from build123d import *

# Parameters (mm, degrees)
BASE_PLATE_DEPTH         = 60
MOUNTING_HOLES_SKETCH_R  = 5
MOUNTING_HOLES_DEPTH     = 60
EYE_UPRIGHT_PROFILE_R    = 12.5
EYE_UPRIGHT_DEPTH        = 10
UPRIGHT_ROOT_FILLET_R6_R = 6


with BuildPart() as part:
    # Base Plate Profile → Base Plate (new body)
    with BuildSketch(Plane.XY):
        Polygon((0, 0), (50, 0), (42, -8), (60, -8), (60, 8), (-60, 8), (-60, -8), (-42, -8), (-50, 0), align=None)
    extrude(amount=-BASE_PLATE_DEPTH)

    # Mounting Holes Sketch → Mounting Holes (cut)
    with BuildSketch(Plane(origin=(0, 8, 0), x_dir=(1, 0, 0), z_dir=(0, 1, 0))):
        with Locations(Location((34, 45, 0), (0, 0, 180))):
            Circle(MOUNTING_HOLES_SKETCH_R)
        with Locations(Location((34, 15, 0), (0, 0, 180))):
            Circle(MOUNTING_HOLES_SKETCH_R)
        with Locations(Location((-34, 45, 0), (0, 0, 180))):
            Circle(MOUNTING_HOLES_SKETCH_R)
        with Locations(Location((-34, 15, 0), (0, 0, 180))):
            Circle(MOUNTING_HOLES_SKETCH_R)
    extrude(amount=-MOUNTING_HOLES_DEPTH, mode=Mode.SUBTRACT)

    # Eye Upright Profile → Eye Upright (add, symmetric)
    with BuildSketch(Plane(origin=(0, 0, 0), x_dir=(0, 0, -1), z_dir=(1, 0, 0))):
        with BuildLine():
            Line((0, 8), (0, 34))
            ThreePointArc((0, 34), (30, 64), (60, 34))
            Line((60, 34), (60, 8))
            Line((60, 8), (0, 8))
        make_face()
        with Locations((30, 34)):
            Circle(EYE_UPRIGHT_PROFILE_R, mode=Mode.SUBTRACT)
    extrude(amount=EYE_UPRIGHT_DEPTH, both=True)

    # Upright Root Fillet R6
    upright_root_fillet_r6_edges = [part.edges().sort_by_distance(p)[0] for p in [
        (-60, 8, -30),
        (60, 8, -30),
        (10, 8, -30),
        (-10, 8, -30),
    ]]
    fillet(upright_root_fillet_r6_edges, radius=UPRIGHT_ROOT_FILLET_R6_R)


solid = part.part
Design review of the part built by this model. Coordinates are the model's own, in mm. A direction names the side the tool comes from. Give positions to 0.01 mm unless a question says otherwise; leave off trailing zeros. Loops run counter-clockwise (first coordinate to the right, second up) from the corner with the lowest first, then second, coordinate; pieces in that order, holes last. Notation, with made-up numbers: M -29,75 L 20,75 A18 ccw 20,80 Z; hole C -33,-38.5 d8. An arc over 180 degrees is marked long. Answer as a JSON object with one key per item and string values.
Item 1: Wall thickness on line 1 along Z through (x, y) = (-34, 2); line 2 along Z through (x, y) = (4.5, 34.5); line 3 along X through (y, z) = (6.5, -18): over which ranges is each line inside the solid? List them lowest first.
Output values:
{"line 1": "z = -60 to -50, -40 to -20, -10 to 0", "line 2": "z = -60 to -42.49, -17.51 to 0", "line 3": "x = -57.97 to -38, -30 to 30, 38 to 57.97"}
Item 2: Mouldability with a two-part tool opening along X and no side actions: class faces 1 (the face through (-60, -3, -30)), 2 (the face through (0.14, 63.993, -29.34)), 3 (the face through (46, -4, -30)), 4 (the face through (-46, -4, -30)) as pulls with the +X half, pulls with the -X half, needs draft (parallel to the pull), parting line crosses it, or undercut.
Output values:
{"face 1": "pulls with the -X half", "face 2": "needs draft", "face 3": "undercut", "face 4": "undercut"}
Item 3: For P1, Ø25, axis at y = 41.5, z = -37, coming from the +X side; P2, Ø3, axis at x = 43.5, z = -31, coming from the +Y side; P3, Ø10, axis at x = 11.5, z = -29, coming from the -Y side; P4, Ø1.5, axis at x = 1, y = 10.5, coming from the +Z side, all flat-tipped, find the tip position at first contact; note any pin that passes through.
Output values:
{"P1": "stops at x = 10", "P2": "stops at y = 8", "P3": "stops at y = 0", "P4": "stops at z = 0"}
Item 4: We need section A-A (z = -30). State the section outline as (x, y) points.
Output values:
{"outline": "M -60,-8 L -42,-8 L -50,0 L 50,0 L 42,-8 L 60,-8 L 60,2 A6 ccw 54,8 L 16,8 A6 cw 10,14 L 10,21.5 L -10,21.5 L -10,14 A6 cw -16,8 L -54,8 A6 ccw -60,2 Z; M -10,46.5 L 10,46.5 L 10,64 L -10,64 Z"}
Item 5: We need section D-D (x = -48). State the section outline as (y, z) points.
Output values:
{"outline": "M -8,-60 L -2,-60 L -2,0 L -8,0 Z; M 0,-60 L 8,-60 L 8,0 L 0,0 Z"}
Item 6: We need section C-C (y = 30.5). State the section outline as (x, z) points, and give its area (3 significant figures).
Output values:
{"outline": "M -10,-60 L 10,-60 L 10,-42 L -10,-42 Z; M -10,-18 L 10,-18 L 10,0 L -10,0 Z", "area": "720 mm2"}
Item 7: Machinability: for faces 5 (the face through (60, -3, -30)), 6 (the face through (10, 45, -37)), 7 (the face through (-1, 0, -30)), 8 (the face through (-35, 8, -30)), 9 (the face through (-30, 4, -42)), which of the approach directions +Z, -Z, +X, -X, +Y, -Y give a long, thin tool a straight path to every point of the face, cutting with its end or side? Answer none if there is none.
Output values:
{"face 5": "+Z, -Z, +X, +Y, -Y", "face 6": "+Z, -Z, +X, +Y", "face 7": "+Z, -Z", "face 8": "+Z, -Z, -X, +Y", "face 9": "+Y, -Y"}
Item 8: We need section B-B (x = -34). State the section outline as (y, z) points.
Output values:
{"outline": "M 0,-60 L 8,-60 L 8,-50 L 0,-50 Z; M 0,-40 L 8,-40 L 8,-20 L 0,-20 Z; M 0,-10 L 8,-10 L 8,0 L 0,0 Z"}
